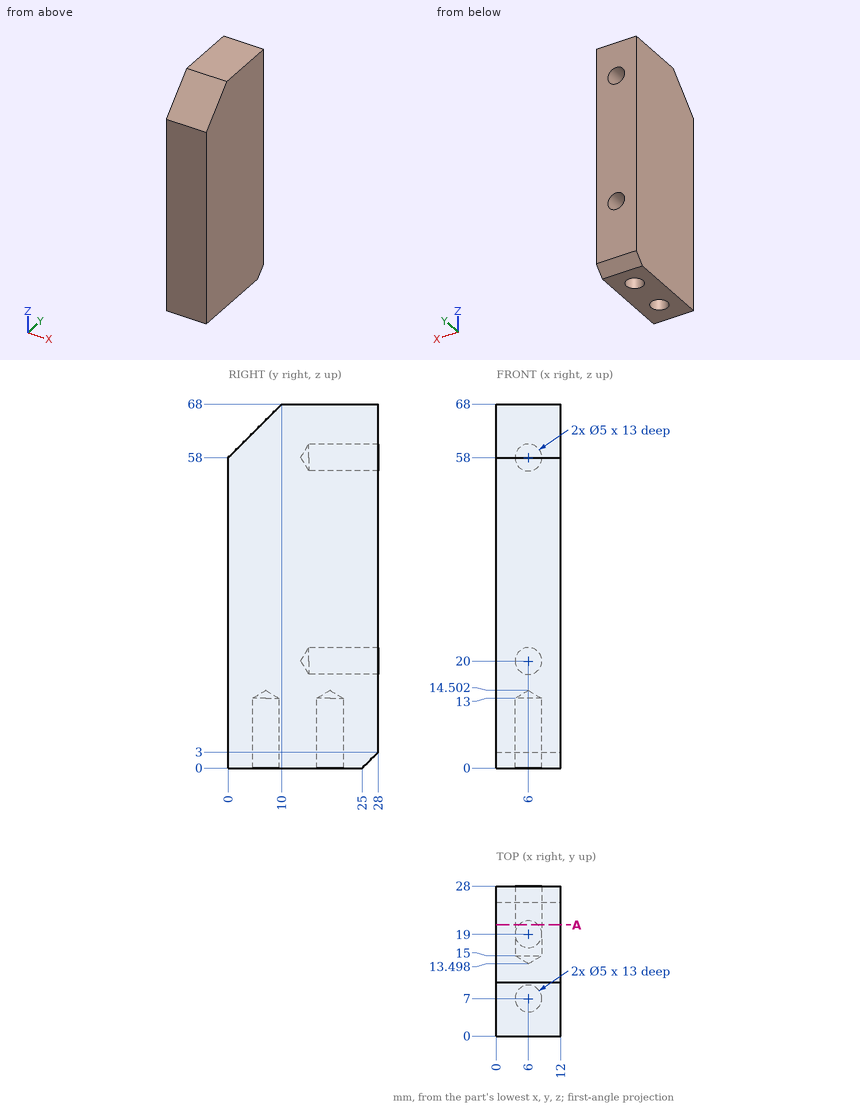
Study the drawing (mm; zero at the part's minimum x, y, z) and answer. Coordinates: 2 decimals unless noted, no trailing zeros. Write each question's results on one line, items separated by ' | '.
Item 1: Consider probe 1 along Z at (x, y) = (6, 24.25); probe 2 along Y at (x, z) = (6, 5); probe 3 along X at (y, z) = (20.5, 20). Determine where each line is inside the solid, lowest interval first. Write a range as [from, to].
Answer below:
probe 1: [0, 17.5], [22.5, 55.5], [60.5, 68] | probe 2: [0, 4.5], [9.5, 16.5], [21.5, 28] | probe 3: [0, 3.5], [8.5, 12]
Item 2: The part is cut by section A-A on y = 20.75. State how many separate pieces and enclosed holes the cut face has, and give its area (3 significant figures).
Answer below:
separate pieces: 1 | enclosed holes: 2 | area: 729 mm2
Item 3: Given P1, Ø4, axis at x = 6, z = 58, coming from the +Y side; P2, Ø4.5, axis at x = 6, y = 7, coming from the -Z side, each flat-ended and moving along its own axis, determine where each tip first touches the part or whether it passes through.
Answer below:
P1: y = 14.7 | P2: z = 13.15
